```python
from build123d import *

# Parameters (mm, degrees)
BOSS_EXTRUDE1_DEPTH = 0.8


with BuildPart() as part:
    # Sketch1 → Boss-Extrude1 (new body)
    with BuildSketch(Plane.XY):
        with BuildLine():
            Line((-0.44416607, 3.673243322), (-0.44416607, 6.097784133))
            Line((-0.44416607, 6.097784133), (-2.402419126, 6.097784133))
            Line((-2.402419126, 6.097784133), (-2.402419126, 4.027962555))
            ThreePointArc((-2.402419126, 4.027962555), (-0.000948808, -4.689999904), (2.404048678, 4.026990186))
            Line((2.404048678, 4.026990186), (2.404048678, 6.097784133))
            Line((2.404048678, 6.097784133), (0.479079413, 6.097784133))
            Line((0.479079413, 6.097784133), (0.479079413, 3.668853079))
            ThreePointArc((0.479079413, 3.668853079), (-0.017594145, -3.699958168), (-0.44416607, 3.673243322))
        make_face()
    extrude(amount=BOSS_EXTRUDE1_DEPTH)


solid = part.part
```
Source: CAD feature listing. Evaluate the final solid. Frame: model axes, mm. Coordinates: 2 decimals unless noted, no trailing zeros. Loops run counter-clockwise (first coordinate to the right, second up) from the corner with the lowest first, then second, coordinate; pieces in that order, holes last. Notation, with made-up numbers: M -9,27 L 19,27 A18 ccw 19,32 Z; hole C 3.25,-16 d1. An arc over 180 degrees is marked long. Use CSV: the item, a comma, the result in double quotes.
(1) Line query: line 1 (X direction, y = 5.5, z = 0.15); line 2 (X direction, y = 0, z = 0.3); line 3 (Y direction, x = -3.25, z = 0.6). Output: solid intervals per line, ascending. Write a range as [from, to].
Answers follow:
line 1,"[-2.4, -0.44], [0.48, 2.4]"
line 2,"[-4.69, -3.7], [3.7, 4.69]"
line 3,"[-3.38, -1.77], [1.77, 3.38]"
(2) Cut plane A-A on y = 0. Return loops of the section in (x, z).
Answers follow:
outline,"M -4.69,0 L -3.7,0 L -3.7,0.8 L -4.69,0.8 Z; M 3.7,0 L 4.69,0 L 4.69,0.8 L 3.7,0.8 Z"
(3) Draft query along X for faces 1 (the face through (-0.172, -4.687, 0.394)), 2 (the face through (2, 4, 0)), 3 (the face through (0.1, -3.7, 0.4)). Return one class per face: pulls with the +X half, pulls with the -X half, needs draft (parallel to the pull), parting line crosses it, or undercut.
Answers follow:
face 1,"parting line crosses it"
face 2,"needs draft"
face 3,"undercut"
(4) Cut plane D-D on x = 0. Return loops of the section in (y, z).
Answers follow:
outline,"M -4.69,0 L -3.7,0 L -3.7,0.8 L -4.69,0.8 Z"
(5) Cut plane B-B on x = -3. Return loops of the section in (y, z), and give its area (3 significant figures).
Answers follow:
outline,"M -3.61,0 L -2.17,0 L -2.17,0.8 L -3.61,0.8 Z; M 2.17,0 L 3.61,0 L 3.61,0.8 L 2.17,0.8 Z"
area,"2.30 mm²"
(6) Cut plane C-C on z = 0.35. Return loops of the section in (x, y), and give its area (3 significant figures).
Answers follow:
outline,"M -2.4,4.03 A4.69 ccw long 2.4,4.03 L 2.4,6.1 L 0.48,6.1 L 0.48,3.67 A3.7 cw long -0.44,3.67 L -0.44,6.1 L -2.4,6.1 Z"
area,"31.7 mm²"
(7) Contact query for flat-ended pins moving along their axis: pin 1 (5 mm diameter, centred on x = -3, y = -3, fed in from -Z); pin 2 (4.5 mm diameter, centred on x = 0, y = 0, fed in from +Z). Output: stop coordinate, or through.
Answers follow:
pin 1,"z = 0"
pin 2,"through"
